Print and shaded views of the part. All mm, measured from the part's lowest x, y and z. A direction names the side the tool comes from. Give positions to 0.01 mm unless a question says otherwise; leave off trailing zeros. Loops run counter-clockwise (first coordinate to the right, second up) from the corner with the lowest first, then second, coordinate; pieces in that order, holes last. Notation, with made-up numbers: M 69,-1 L 94,-1 A30 ccw 94,31 Z; hole C -31,13 d11. An arc over 180 degrees is marked long. Answer as CSV lines item,"result".
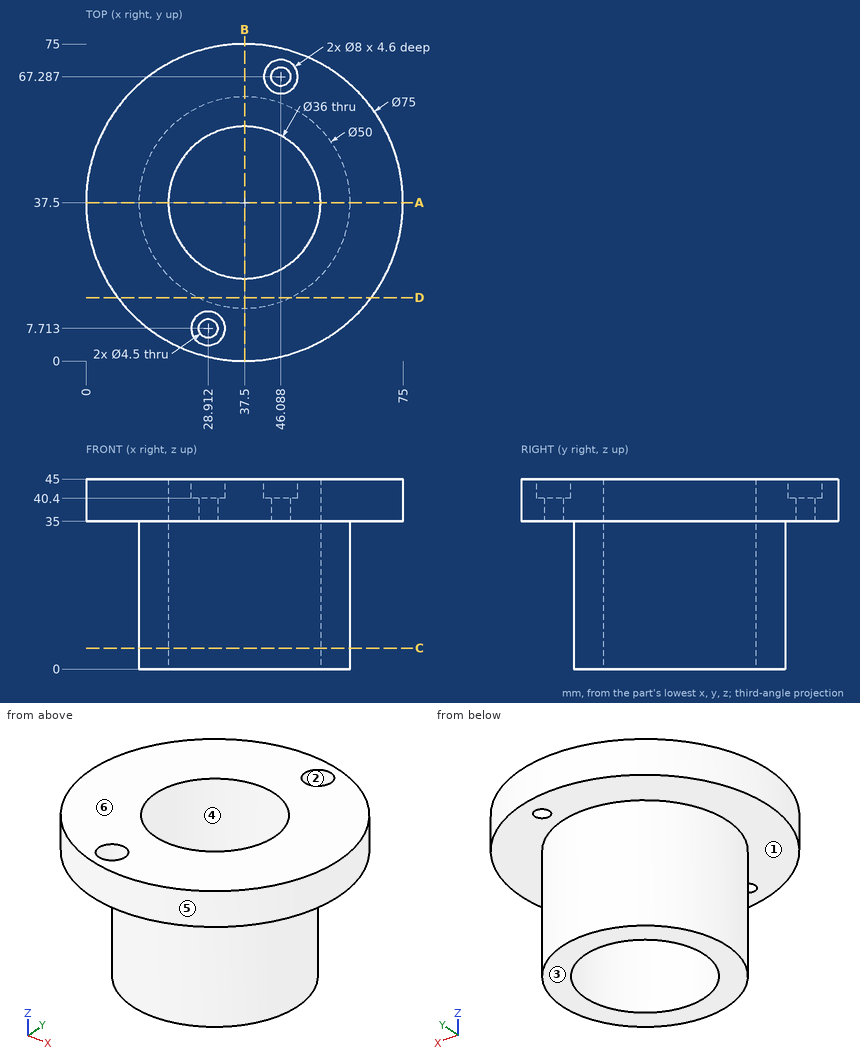
Q1. Mould opens along X. For the marked faces 4, 5 and 6 say: released by +X, released by -X, zero draft, split by the parting line, or undercut.
Solution:
face 4,"undercut"
face 5,"split by the parting line"
face 6,"zero draft"
Q2. Pin check, flat tips, straight feed: P1, Ø6, axis at x = 28.91, y = 7.71, coming from the +Z side; P2, Ø6, axis at x = 63.5, z = 6, coming from the -Y side (1 decimal); P3, Ø2, axis at x = 46, z = 40, coming from the -Y side. Stop position of each tip, or through.
Solution:
P1,"stops at z = 40.4"
P2,"stops at y = 27.7"
P3,"stops at y = 0.76"
Q3. Cut at D-D (y = 15). Write the cut outline in (x, z).
Solution:
outline,"M 7.5,35 L 26.6,35 L 26.6,0 L 48.4,0 L 48.4,35 L 67.5,35 L 67.5,45 L 7.5,45 Z"
Q4. Cut at A-A (y = 37.5). Write the cut outline in (x, z).
Solution:
outline,"M 0,35 L 12.5,35 L 12.5,0 L 19.5,0 L 19.5,45 L 0,45 Z; M 55.5,0 L 62.5,0 L 62.5,35 L 75,35 L 75,45 L 55.5,45 Z"
Q5. Cut at C-C (z = 5). Write the cut outline in (x, y).
Solution:
outline,"C 37.5,37.5 d50; hole C 37.5,37.5 d36"
Q6. Which spindle directions (+Z, -Z, +X, -X, +Y, -Y) get a long thin tool onto all of the face, cutting with end or side? Do the marked faces 1, 2 and 3. Say none if no direction does.
Solution:
face 1,"-Z"
face 2,"+Z"
face 3,"-Z, +X, -X, +Y, -Y"
Q7. Wall check: line 1 (Y direction, x = 38, z = 39.5); line 2 (Z direction, x = 38.5, y = 3); line 3 (Y direction, x = 24, z = 11.5) (1 decimal). Give the ranges that are in metal, low to high. Write a range as [from, to].
Solution:
line 1,"y = [0, 19.51], [55.49, 75]"
line 2,"z = [35, 45]"
line 3,"y = [16.5, 25.6], [49.4, 58.5]"
